```python
from build123d import *

# Parameters (mm, degrees)
SKETCH1_W           = 80
SKETCH1_H           = 12
BOSS_EXTRUDE1_DEPTH = 8
CHAMFER1_SIZE       = 2
SKETCH2_R           = 2.25
CUT_EXTRUDE1_DEPTH  = 10
CUT_EXTRUDE2_DEPTH  = 10


with BuildPart() as part:
    # Sketch1 → Boss-Extrude1 (new body)
    with BuildSketch(Plane(origin=(0, 0, 0), x_dir=(1, 0, 0), z_dir=(0, 1, 0))):
        with Locations((40, 6)):
            Rectangle(SKETCH1_W, SKETCH1_H)
    extrude(amount=BOSS_EXTRUDE1_DEPTH)

    # Chamfer1
    chamfer1_edges = [part.edges().sort_by_distance(p)[0] for p in [
        (0, 4, -12),
        (80, 4, -12),
        (80, 4, 0),
        (0, 4, 0),
    ]]
    chamfer(chamfer1_edges, length=CHAMFER1_SIZE)

    # Sketch2 → Cut-Extrude1 (cut)
    with BuildSketch(Plane.XZ):
        with Locations(Location((10, -6, 0), (0, 0, 270))):
            Circle(SKETCH2_R)
        with Locations(Location((70, -6, 0), (0, 0, 270))):
            Circle(SKETCH2_R)
    extrude(amount=-CUT_EXTRUDE1_DEPTH, mode=Mode.SUBTRACT)

    # Sketch4 → Cut-Extrude2 (cut)
    with BuildSketch(Plane.XZ):
        with BuildLine():
            Line((7.75, -8.25), (7.75, -3.75))
            ThreePointArc((7.75, -3.75), (10, -1.5), (12.25, -3.75))
            Line((12.25, -3.75), (12.25, -8.25))
            ThreePointArc((12.25, -8.25), (10, -10.5), (7.75, -8.25))
        make_face()
        with BuildLine():
            Line((72.25, -8.25), (72.25, -3.75))
            ThreePointArc((72.25, -3.75), (70, -1.5), (67.75, -3.75))
            Line((67.75, -3.75), (67.75, -8.25))
            ThreePointArc((67.75, -8.25), (70, -10.5), (72.25, -8.25))
        make_face()
    extrude(amount=-CUT_EXTRUDE2_DEPTH, mode=Mode.SUBTRACT)


solid = part.part
```
Verification items for the finished model (mm, model axes). A direction names the side the tool comes from. Coordinates: 2 decimals unless noted, no trailing zeros. Loops run counter-clockwise (first coordinate to the right, second up) from the corner with the lowest first, then second, coordinate; pieces in that order, holes last. Notation, with made-up numbers: (-16, 41) - (-5, 41) arc R11 ccw to (-5, 56) - close; hole circle Ø1 at (-5, -1.5). An arc over 180 degrees is marked (long way). Return JSON: item names as keys, results as strings.
1. Section check A-A, the plane x = 70. Record the boundary of the cut face in (y, z), then the cut area to 3 significant figures.
Established:
{"outline": "(0, -12) - (8, -12) - (8, -10.5) - (0, -10.5) - close; (0, -1.5) - (8, -1.5) - (8, 0) - (0, 0) - close", "area": "24.0 mm2"}
2. Section check B-B, the plane z = -4.5. Record the boundary of the cut face in (x, y), then the cut area to 3 significant figures.
Established:
{"outline": "(0, 0) - (7.75, 0) - (7.75, 8) - (0, 8) - close; (12.25, 0) - (67.75, 0) - (67.75, 8) - (12.25, 8) - close; (72.25, 0) - (80, 0) - (80, 8) - (72.25, 8) - close", "area": "568 mm2"}
3. Tool access check on faces 5 (the flat face through (72.25, 4, -6)), 6 (the flat face through (79, 4, -1)). Record the directions out of +Z, -Z, +X, -X, +Y, -Y that give a thin tool (end or side, any length) a straight path to the whole face; none if there is none.
Established:
{"face 5": "+Y, -Y", "face 6": "+Z, +X, +Y, -Y"}
4. Section check C-C, the plane y = 5.25. Record the boundary of the cut face in (x, z), then the cut area to 3 significant figures.
Established:
{"outline": "(0, -10) - (2, -12) - (78, -12) - (80, -10) - (80, -2) - (78, 0) - (2, 0) - (0, -2) - close; hole (7.75, -8.25) arc R2.25 ccw to (12.25, -8.25) - (12.25, -3.75) arc R2.25 ccw to (7.75, -3.75) - close; hole (67.75, -8.25) arc R2.25 ccw to (72.25, -8.25) - (72.25, -3.75) arc R2.25 ccw to (67.75, -3.75) - close", "area": "880 mm2"}
5. Thickness scan on L1, parallel to X at y = 7.75, z = -7.75; L2, parallel to X at y = 2, z = -10; L3, parallel to X at y = 5.25, z = -11.5. Record the ranges inside material, lowest first.
Established:
{"L1": "x = 0 to 7.75, 12.25 to 67.75, 72.25 to 80", "L2": "x = 0 to 8.59, 11.41 to 68.59, 71.41 to 80", "L3": "x = 1.5 to 78.5"}
6. Mould release check, pull along X, two halves, no side actions. Record for faces 1 (the flat face through (80, 4, -6)), 2 (the flat face through (1, 4, -1)), 3 (the cylindrical face through (70, 3.9, -10.5)), 4 (the flat face through (7.75, 4, -6)): +X half, -X half, draft (parallel to the pull), parting line (faces both ways), or undercut.
Established:
{"face 1": "+X half", "face 2": "-X half", "face 3": "undercut", "face 4": "undercut"}
